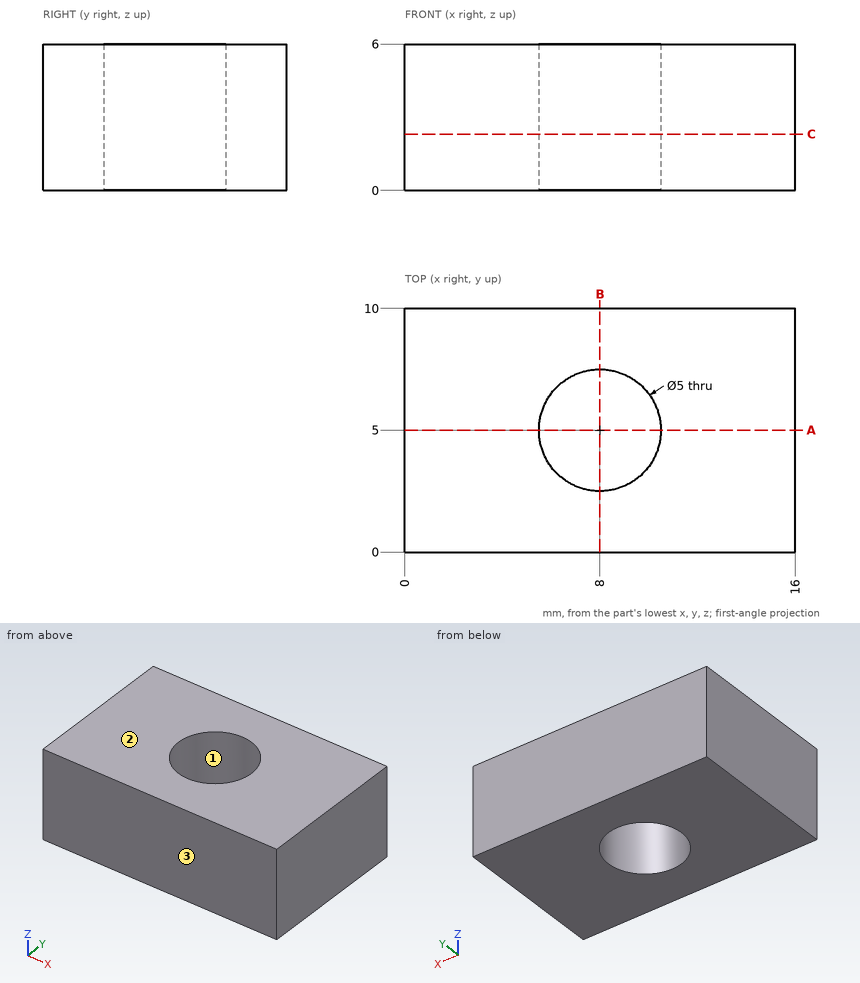
Answer from the drawing. Dimensions are ordinates in mm from the lowest x, y and z of the part. Coordinates: 2 decimals unless noted, no trailing zeros. Order: outer loops, then holes, each group sorted by start corner. A loop starts at its lowest first (then second) coordinate and runs counter-clockwise, first axis right, second up. Notation, with made-up numbers: M 48.5,35 L 100.5,35 A18 ccw 100.5,48 Z; hole C -36,63.5 d7. An arc over 180 degrees is marked long. Put each result on its own line as item: value. Start each with the question number.
Item 1: Given pin 1 Ø3 at (x, y) = (8, 5) entering from -Z, flat-ended and moving along its own axis, determine where the tip first touches the part or whether it passes through.
Item 2: Section A-A, the plane y = 5 is taken. Determine the outline of the cut face in (x, z), plus the area to 3 significant figures.
Item 3: Consider probe 1 along X at (y, z) = (3.5, 1.15); probe 2 along Y at (x, z) = (8, 2.1); probe 3 along X at (y, z) = (7, 5.1). Determine where each line is inside the solid, lowest interval first. Write a range as [from, to].
Item 4: The mould has two halves that part along Y. Classify the marked faces 1, 2 and 3: +Y half, -Y half, draft (parallel to the pull), parting line (faces both ways), or undercut.
Item 5: Section B-B, the plane x = 8 is taken. Determine the outline of the cut face in (y, z).
Item 6: Section C-C, the plane z = 2.3 is taken. Determine the outline of the cut face in (x, y).
Computed:
1. pin 1: passes through
2. outline: M 0,0 L 5.5,0 L 5.5,6 L 0,6 Z; M 10.5,0 L 16,0 L 16,6 L 10.5,6 Z
2. area: 66.0 mm2
3. probe 1: x = [0, 6], [10, 16]
3. probe 2: y = [0, 2.5], [7.5, 10]
3. probe 3: x = [0, 6.5], [9.5, 16]
4. face 1: undercut
4. face 2: draft
4. face 3: -Y half
5. outline: M 0,0 L 2.5,0 L 2.5,6 L 0,6 Z; M 7.5,0 L 10,0 L 10,6 L 7.5,6 Z
6. outline: M 0,0 L 16,0 L 16,10 L 0,10 Z; hole C 8,5 d5
